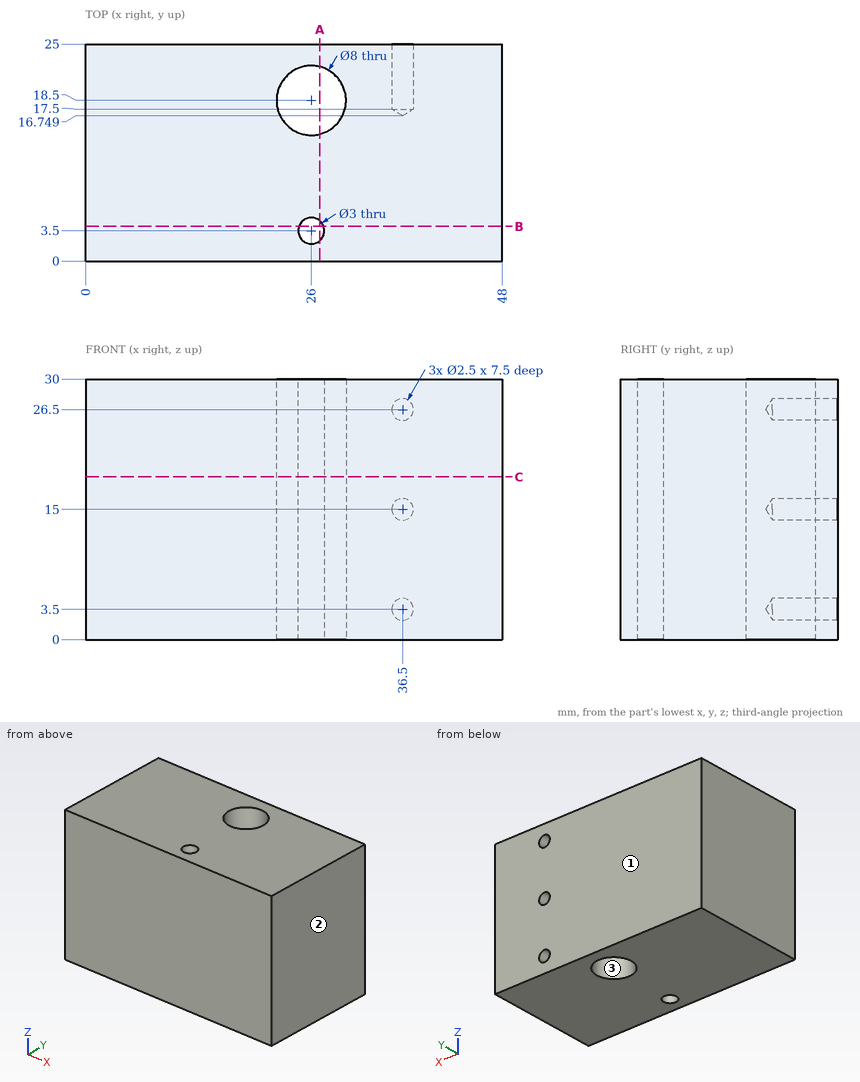
Design review of the part shown in the three views and the two pictorial views. Dimensions are in mm from the part's minimum x, y and z. Coordinates: 2 decimals unless noted, no trailing zeros. Order: outer loops, then holes, each group sorted by start corner. A loop starts at its lowest first (then second) coordinate and runs counter-clockwise, first axis right, second up. Notation, with made-up numbers: (-12, 78.5) -> (46, 78.5) arc R17 ccw to (46, 89.5) -> close; hole circle Ø11 at (21.25, 79.25). An arc over 180 degrees is marked (long way). Use one line per item in the form item = value. Start each with the question number.
(1) Add section A-A on x = 27. State the section outline as (y, z) points, plus the area to 3 significant figures.
(2) Add section B-B on y = 4. State the section outline as (x, z) points, plus the area to 3 significant figures.
(3) Insertion check: pin 1 (1.5 mm diameter, centred on x = 36.5, z = 3.5, fed in from +Y); pin 2 (7 mm diameter, centred on x = 26, y = 18.5, fed in from -Z). Each pin has a flat end and moves straight along its axis. Give the tip position at first contact, or say it passes through.
(4) For probe 1 along Z at (x, y) = (36.5, 21.5); probe 2 along Y at (x, z) = (26, 17.25); probe 3 along X at (y, z) = (20.25, 3.5), list the stretches that pass through material, from the lowest coordinate up.
(5) The part is to be moulded in two halves that separate along X. For the marked faces 1, 2 and 3, say which applies: +X half, -X half, draft (parallel to the pull), parting line (faces both ways), or undercut.
(6) Add section C-C on z = 18.75. State the section outline as (x, y) points, plus the area to 3 significant figures.
Answer block:
q1.outline = (0, 0) -> (2.38, 0) -> (2.38, 30) -> (0, 30) -> close; (4.62, 0) -> (14.63, 0) -> (14.63, 30) -> (4.62, 30) -> close; (22.37, 0) -> (25, 0) -> (25, 30) -> (22.37, 30) -> close
q1.area = 451 mm²
q2.outline = (0, 0) -> (24.59, 0) -> (24.59, 30) -> (0, 30) -> close; (27.41, 0) -> (48, 0) -> (48, 30) -> (27.41, 30) -> close
q2.area = 1,360 mm²
q3.pin_1 = 17.2
q3.pin_2 = through
q4.probe_1 = 0 to 2.25, 4.75 to 13.75, 16.25 to 25.25, 27.75 to 30
q4.probe_2 = 0 to 2, 5 to 14.5, 22.5 to 25
q4.probe_3 = 0 to 22.4, 29.6 to 35.25, 37.75 to 48
q5.face_1 = draft
q5.face_2 = +X half
q5.face_3 = undercut
q6.outline = (0, 0) -> (48, 0) -> (48, 25) -> (0, 25) -> close; hole circle Ø8 at (26, 18.5); hole circle Ø3 at (26, 3.5)
q6.area = 1,140 mm²
